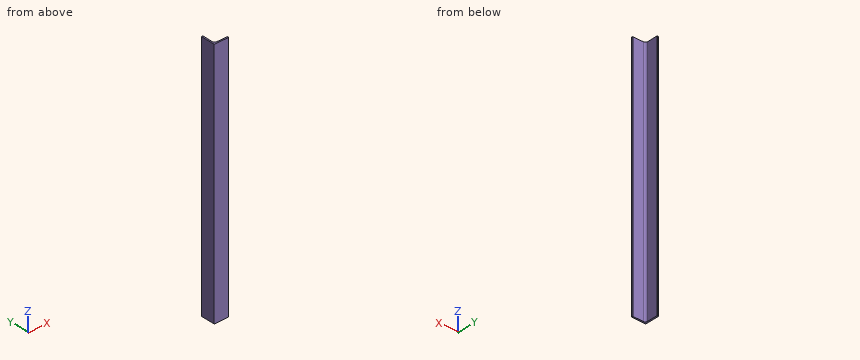
```python
from build123d import *

# Parameters (mm, degrees)
BOSS_EXTRUDE1_DEPTH = 257.5


with BuildPart() as part:
    # Sketch1 → Boss-Extrude1 (new, symmetric)
    with BuildSketch(Plane.XY):
        with BuildLine():
            Line((0, 0), (0, 30))
            Line((0, 30), (2, 30))
            ThreePointArc((2, 30), (2.707106781, 29.707106781), (3, 29))
            Line((3, 29), (3, 7.5))
            ThreePointArc((3, 7.5), (4.318019485, 4.318019485), (7.5, 3))
            Line((7.5, 3), (29, 3))
            ThreePointArc((29, 3), (29.707106781, 2.707106781), (30, 2))
            Line((30, 2), (30, 0))
            Line((30, 0), (0, 0))
        make_face()
    extrude(amount=BOSS_EXTRUDE1_DEPTH, both=True)


solid = part.part
```
The listing builds one solid part. Answer for the finished solid, in the listing's coordinates (mm). Give positions to 0.01 mm unless a question says otherwise; leave off trailing zeros. Order: outer loops, then holes, each group sorted by start corner. A loop starts at its lowest first (then second) coordinate and runs counter-clockwise, first axis right, second up. Notation, with made-up numbers: (-13.5, -10) -> (42.5, -10) arc R28 cw to (42.5, 21) -> close; hole circle Ø5 at (76, 66). An arc over 180 degrees is marked (long way). Answer as CSV lines item,"result". Start each with the question number.
Q1. A cutting plane is placed at B-B (y = 19). Determine the outline of the cut face in (x, z), then the cut area to 4 significant figures.
Q2. A cutting plane is placed at A-A (z = -103). Determine the outline of the cut face in (x, y).
Q3. Find the intervals of material crossed by L1, parallel to Y at x = 25.5, z = -210.5; L2, parallel to Y at x = 4.75, z = -36, in increasing order.
Q4. Given pin 1 (6.5 mm diameter, centred on y = 17.5, z = 123.5, fed in from +X); pin 2 (5 mm diameter, centred on y = 7, z = -178, fed in from +X); pin 3 (11 mm diameter, centred on x = 23.5, z = 81.5, fed in from +Y), each flat-ended and moving along its own axis, determine where each tip first touches the part or whether it passes through.
Results found:
1,outline,"(0, -257.5) -> (3, -257.5) -> (3, 257.5) -> (0, 257.5) -> close"
1,area,"1,545 mm2"
2,outline,"(0, 0) -> (30, 0) -> (30, 2) arc R1 ccw to (29, 3) -> (7.5, 3) arc R4.5 cw to (3, 7.5) -> (3, 29) arc R1 ccw to (2, 30) -> (0, 30) -> close"
3,L1,"0 to 3"
3,L2,"0 to 3.94"
4,pin 1,"x = 3"
4,pin 2,"x = 4.15"
4,pin 3,"y = 3"
